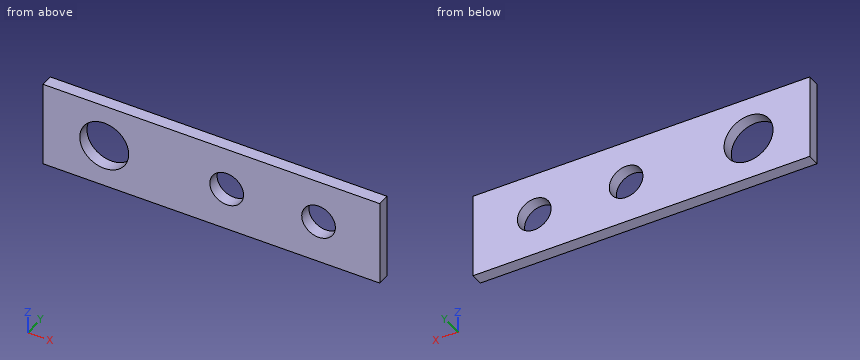
from build123d import *

# Parameters (mm, degrees)
EXTRUDE_1_DEPTH      = 1
EXTRUDE_1_DEPTH_BACK = 1
SKETCH_1_W           = 55
SKETCH_1_H           = 14
SKETCH_1_R           = 2.75
SKETCH_1_R_2         = 4


with BuildPart() as part:
    # 草图1 → 凸台-拉伸1 (new, two sides: drawn at the far end of the back side and taken through both)
    with BuildSketch(Plane(origin=(0, 0, 0), x_dir=(1, 0, 0), z_dir=(0, 1, 0)).offset(-EXTRUDE_1_DEPTH_BACK)):
        with Locations((17.5, 0)):
            Rectangle(SKETCH_1_W, SKETCH_1_H)
        with Locations(Location((35, 0, 0), (0, 0, 270))):
            Circle(SKETCH_1_R, mode=Mode.SUBTRACT)
        with Locations(Location((20, 0, 0), (0, 0, 270))):
            Circle(SKETCH_1_R, mode=Mode.SUBTRACT)
        with Locations(Location((0, 0, 0), (0, 0, 270))):
            Circle(SKETCH_1_R_2, mode=Mode.SUBTRACT)
    extrude(amount=EXTRUDE_1_DEPTH + EXTRUDE_1_DEPTH_BACK)


solid = part.part
Input: part model. Units: mm. Frame: model coordinates. Coordinates: 2 decimals unless noted, no trailing zeros. Order: outer loops, then holes, each group sorted by start corner. A loop starts at its lowest first (then second) coordinate and runs counter-clockwise, first axis right, second up. Notation, with made-up numbers: M -19,63.5 L 0,63.5 A33 cw 0,99.5 Z; hole C 11.25,54 d10. An arc over 180 degrees is marked long. Answer in a Markdown table with one row per item.
(1) Section query A-A, the plane z = 0. Output: boundary loops of the cut face in (x, y), plus the area to 3 significant figures.
Numbers:
| item | result |
|---|---|
| outline | M -10,-1 L -4,-1 L -4,1 L -10,1 Z; M 4,-1 L 17.25,-1 L 17.25,1 L 4,1 Z; M 22.75,-1 L 32.25,-1 L 32.25,1 L 22.75,1 Z; M 37.75,-1 L 45,-1 L 45,1 L 37.75,1 Z |
| area | 72.0 mm^2 |
(2) Section query C-C, the plane x = 0. Output: boundary loops of the cut face in (y, z).
Numbers:
| item | result |
|---|---|
| outline | M -1,-7 L 1,-7 L 1,-4 L -1,-4 Z; M -1,4 L 1,4 L 1,7 L -1,7 Z |
(3) Section query B-B, the plane x = 20. Output: boundary loops of the cut face in (y, z).
Numbers:
| item | result |
|---|---|
| outline | M -1,-7 L 1,-7 L 1,-2.75 L -1,-2.75 Z; M -1,2.75 L 1,2.75 L 1,7 L -1,7 Z |
(4) Section query D-D, the plane z = -2.25. Output: boundary loops of the cut face in (x, y).
Numbers:
| item | result |
|---|---|
| outline | M -10,-1 L -3.31,-1 L -3.31,1 L -10,1 Z; M 3.31,-1 L 18.42,-1 L 18.42,1 L 3.31,1 Z; M 21.58,-1 L 33.42,-1 L 33.42,1 L 21.58,1 Z; M 36.58,-1 L 45,-1 L 45,1 L 36.58,1 Z |
(5) Material intervals for line 1 (X direction, y = -0.2, z = 0); line 2 (X direction, y = 0.1, z = 2.25); line 3 (X direction, y = 0.15, z = 3.5), sorted ascending. Write a range as [from, to].
Numbers:
| item | result |
|---|---|
| line 1 | x = [-10, -4], [4, 17.25], [22.75, 32.25], [37.75, 45] |
| line 2 | x = [-10, -3.31], [3.31, 18.42], [21.58, 33.42], [36.58, 45] |
| line 3 | x = [-10, -1.94], [1.94, 45] |
